```python
from build123d import *

# Parameters (mm, degrees)
SKETCH1_W                                         = 110
SKETCH1_H                                         = 350
BOSS_EXTRUDE1_DEPTH                               = 10
HOLE_SIZE_BY_SOCKET_HEAD_CAP_SCREW_TY_D           = 5.5
HOLE_SIZE_BY_SOCKET_HEAD_CAP_SCREW_TY_CBORE_D     = 10
HOLE_SIZE_BY_SOCKET_HEAD_CAP_SCREW_TY_CBORE_DEPTH = 5.7
HOLE_SIZE_BY_SOCKET_HEAD_CAP_SCRE_2_D             = 6.6
HOLE_SIZE_BY_SOCKET_HEAD_CAP_SCRE_2_CBORE_D       = 11
HOLE_SIZE_BY_SOCKET_HEAD_CAP_SCRE_2_CBORE_DEPTH   = 6.8
CHAMFER1_SIZE                                     = 2
HOLE_SIZE_BY_SOCKET_HEAD_CAP_SCRE_3_D             = 6.6
HOLE_SIZE_BY_SOCKET_HEAD_CAP_SCRE_3_CBORE_D       = 11
HOLE_SIZE_BY_SOCKET_HEAD_CAP_SCRE_3_CBORE_DEPTH   = 6.8
SKETCH8_R                                         = 16.5
CUT_EXTRUDE1_DEPTH                                = 184.711730709
M5_TAPPED_HOLE1_D                                 = 4.2
SKETCH11_R                                        = 15
CUT_EXTRUDE2_DEPTH                                = 184.711730709


with BuildPart() as part:
    # Sketch1 → Boss-Extrude1 (new body)
    with BuildSketch(Plane(origin=(0, 0, 0), x_dir=(1, 0, 0), z_dir=(0, 1, 0))):
        Rectangle(SKETCH1_W, SKETCH1_H)
    extrude(amount=BOSS_EXTRUDE1_DEPTH)

    # Hole Size _ by_ Socket Head Cap Screw Ty (through all)
    with Locations(Plane.XZ):
        with Locations((-18, 131.5), (18, 131.5), (18, 163.5), (-18, 163.5), (-18, -163.5), (-18, -131.5), (18, -163.5), (18, -131.5)):
            CounterBoreHole(HOLE_SIZE_BY_SOCKET_HEAD_CAP_SCREW_TY_D / 2, HOLE_SIZE_BY_SOCKET_HEAD_CAP_SCREW_TY_CBORE_D / 2, HOLE_SIZE_BY_SOCKET_HEAD_CAP_SCREW_TY_CBORE_DEPTH)

    # Hole Size _ by_ Socket Head Cap Scre 2 (through all)
    with Locations(Plane.XZ):
        with Locations((-17, -17), (17, -17), (17, 17), (-17, 17)):
            CounterBoreHole(HOLE_SIZE_BY_SOCKET_HEAD_CAP_SCRE_2_D / 2, HOLE_SIZE_BY_SOCKET_HEAD_CAP_SCRE_2_CBORE_D / 2, HOLE_SIZE_BY_SOCKET_HEAD_CAP_SCRE_2_CBORE_DEPTH)

    # Chamfer1
    chamfer1_edges = [part.edges().sort_by_distance(p)[0] for p in [
        (55, 5, 175),
        (-55, 5, 175),
        (-55, 5, -175),
        (55, 5, -175),
    ]]
    chamfer(chamfer1_edges, length=CHAMFER1_SIZE)

    # Hole Size _ by_ Socket Head Cap Scre 3 (through all)
    with Locations(Plane(origin=(0, 0, 0), x_dir=(-1, 0, 0), z_dir=(0, -1, 0))):
        with Locations((30, 35), (-30, 35)):
            CounterBoreHole(HOLE_SIZE_BY_SOCKET_HEAD_CAP_SCRE_3_D / 2, HOLE_SIZE_BY_SOCKET_HEAD_CAP_SCRE_3_CBORE_D / 2, HOLE_SIZE_BY_SOCKET_HEAD_CAP_SCRE_3_CBORE_DEPTH)

    # Sketch8 → Cut-Extrude1 (cut, through all)
    with BuildSketch(Plane.XZ):
        with Locations(Location((0, -80, 0), (0, 0, 270))):
            Circle(SKETCH8_R)
        with Locations(Location((0, 80, 0), (0, 0, 270))):
            Circle(SKETCH8_R)
    extrude(amount=-CUT_EXTRUDE1_DEPTH, mode=Mode.SUBTRACT)

    # M5 Tapped Hole1 (through all)
    with Locations(Plane(origin=(0, 10, 0), x_dir=(1, 0, 0), z_dir=(0, 1, 0))):
        with Locations((-15.202795796, 95.202795796), (15.202795796, 64.797204204), (-15.202795796, 64.797204204), (15.202795796, 95.202795796), (-15.202795796, -64.797204204), (15.202795796, -95.202795796), (15.202795796, -64.797204204), (-15.202795796, -95.202795796)):
            Hole(M5_TAPPED_HOLE1_D / 2)

    # Sketch11 → Cut-Extrude2 (cut, through all)
    with BuildSketch(Plane(origin=(0, 10, 0), x_dir=(1, 0, 0), z_dir=(0, 1, 0))):
        with Locations(Location((0, 0, 0), (0, 0, 270))):
            Circle(SKETCH11_R)
    extrude(amount=-CUT_EXTRUDE2_DEPTH, mode=Mode.SUBTRACT)


solid = part.part
```
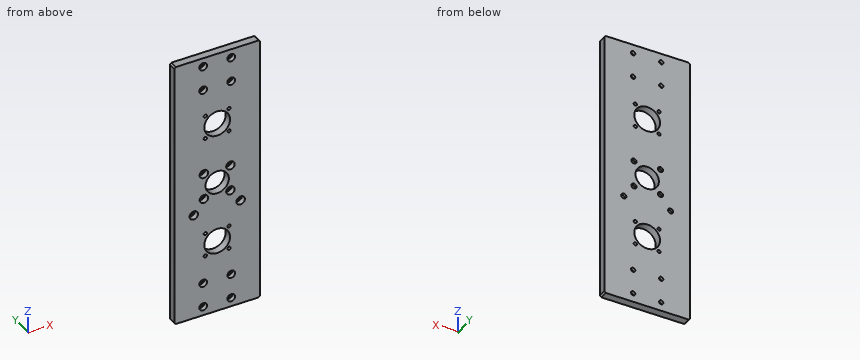
Input: part model. Units: mm. Frame: model coordinates. Coordinates: 2 decimals unless noted, no trailing zeros. Loops run counter-clockwise (first coordinate to the right, second up) from the corner with the lowest first, then second, coordinate; pieces in that order, holes last.
Q1. Section B-B, the plane x = -30. Return the cut outline in (y, z), and give its area (3 significant figures).
Results are:
outline: (0, -175) - (10, -175) - (10, -38.3) - (6.8, -38.3) - (6.8, -40.5) - (0, -40.5) - close; (0, -29.5) - (6.8, -29.5) - (6.8, -31.7) - (10, -31.7) - (10, 175) - (0, 175) - close
area: 3,400 mm2
Q2. Contact query for flat-ended pins moving along their axis: pin 1 (16 mm diameter, centred on x = -18, z = -163.5, fed in from +Y); pin 2 (5 mm diameter, centred on x = -16, z = 132.5, fed in from -Y). Output: stop coordinate, or through.
Results are:
pin 1: stops at y = 10
pin 2: stops at y = 5.7
Q3. Section D-D, the plane z = -80. Return the cut outline in (x, y).
Results are:
outline: (-55, 0) - (-16.5, 0) - (-16.5, 10) - (-55, 10) - close; (16.5, 0) - (55, 0) - (55, 10) - (16.5, 10) - close
Q4. Line query: line 1 along Z through (x, y) = (-30.5, 2.25); line 2 along Z through (x, y) = (-30, 9.3); line 3 along Z through (x, y) = (11.5, 9.25). Output: solid intervals per line, ascending.
Results are:
line 1: z = -175 to -40.48, -29.52 to 175
line 2: z = -175 to -38.3, -31.7 to 175
line 3: z = -175 to -91.83, -68.17 to -9.63, 9.63 to 68.17, 91.83 to 175
Q5. Section A-A, the plane z = 0. Return the cut outline in (x, y).
Results are:
outline: (-55, 0) - (-15, 0) - (-15, 10) - (-55, 10) - close; (15, 0) - (55, 0) - (55, 10) - (15, 10) - close
Q6. Section C-C, the plane y = 1.5. Give the number of separate pieces and of enclosed holes in the cut face, and give its area (3 significant figures).
Results are:
separate pieces: 1
enclosed holes: 25
area: 34,800 mm2
